Source: CAD feature listing. Evaluate the final solid. Frame: model axes, mm. A direction names the side the tool comes from. Round coordinates to 2 decimals unless told otherwise and drop trailing zeros. Write each loop counter-clockwise with the first axis right and the second up, starting at its lowest first coordinate (ties: lowest second). Pieces come first, ordered by that corner, then holes. Notation, with made-up numbers: M 7,-5.75 L 60,-5.75 A24 cw 60,24.25 Z; hole C 60.25,-7.5 d2. An arc over 180 degrees is marked long. Answer in a Markdown table with one row per item. Add a question column.
Item 1: Cut plane A-A on y = 2.25. Return loops of the section in (x, z), and give its area (3 significant figures).
Item 2: Cut plane B-B on z = -49. Return loops of the section in (x, y).
Item 3: Set-up query: faces 5 (the face through (-0.8, 15.1, -82.4)), 6 (the face through (-41.15, 14.93, -32.74)). Return all of +Z, -Z, +X, -X, +Y, -Y with unobstructed straight access to the full face (end or side cutting, diameter ignored); none if empty.
Item 4: Contact query for flat-ended pins moving along their axis: pin 1 (5 mm diameter, centred on y = 16, z = 35, fed in from -X); pin 2 (9.5 mm diameter, centred on x = 37.5, z = -37.5, fed in from +Y); pin 3 (11 mm diameter, centred on x = -37.5, z = -37.5, fed in from +Y). Output: stop coordinate, or through.
Item 5: Mould query, pull axis Z, two halves, no side actions, for faces 1 (the face through (-62.236, 5.07, -68.494)), 2 (the face through (36.87, 7.02, 36.67)), 3 (the face through (78.945, 5.07, -78.479)), 4 (the face through (-82.4, 15.1, 0.8)). Classes: released by +Z, released by -Z, zero draft, split by the parting line, or undercut.
Item 6: Material intervals for probe 1 along X at (y, z) = (15.75, -37.5); probe 2 along Z at (x, y) = (62.5, 8.25), sorted ascending.
from build123d import *

# Parameters (mm, degrees)
BASE_PLATE_SKETCH_175X175_W = 175
BASE_PLATE_SKETCH_175X175_H = 175
BASE_PLATE_DEPTH            = 20
CORNER_FILLETS_R30_R        = 30
EDGE_CHAMFER_10X45_SIZE     = 10
DOWEL_HOLES_12_INNER_D      = 12
DOWEL_HOLES_12_INNER_DEPTH  = 10
DOWEL_HOLES_12_INNER_TIP    = 3.605163714
DOWEL_HOLES_12_OUTER_D      = 12
DOWEL_HOLES_12_OUTER_DEPTH  = 10
DOWEL_HOLES_12_OUTER_TIP    = 3.605163714


with BuildPart() as part:
    # Base Plate Sketch 175x175 → Base Plate (new body)
    with BuildSketch(Plane(origin=(0, 0, 0), x_dir=(1, 0, 0), z_dir=(0, 1, 0))):
        Rectangle(BASE_PLATE_SKETCH_175X175_W, BASE_PLATE_SKETCH_175X175_H)
    extrude(amount=BASE_PLATE_DEPTH)

    # Corner Fillets R30
    corner_fillets_r30_edges = [part.edges().sort_by_distance(p)[0] for p in [
        (87.5, 10, 87.5),
        (-87.5, 10, 87.5),
        (-87.5, 10, -87.5),
        (87.5, 10, -87.5),
    ]]
    fillet(corner_fillets_r30_edges, radius=CORNER_FILLETS_R30_R)

    # Edge Chamfer 10x45
    edge_chamfer_10x45_edges = [part.edges().sort_by_distance(p)[0] for p in [
        (-87.5, 20, 0),
        (0, 20, -87.5),
        (87.5, 20, 0),
        (0, 20, 87.5),
        (-78.713203436, 20, 78.713203436),
        (78.713203436, 20, 78.713203436),
        (78.713203436, 20, -78.713203436),
        (-78.713203436, 20, -78.713203436),
    ]]
    chamfer(edge_chamfer_10x45_edges, length=EDGE_CHAMFER_10X45_SIZE)

    # Dowel Holes Ø12 Inner
    with Locations(Plane(origin=(-37.5, 20, -37.5), x_dir=(0, 0, 1), z_dir=(0, 1, 0))):
        with Locations((0, 0), (0, 75), (75, 75), (75, 0)):
            Hole(DOWEL_HOLES_12_INNER_D / 2, depth=DOWEL_HOLES_12_INNER_DEPTH)
            with Locations((0, 0, -(DOWEL_HOLES_12_INNER_DEPTH + DOWEL_HOLES_12_INNER_TIP / 2))):  # 118° drill point
                Cone(0, DOWEL_HOLES_12_INNER_D / 2, DOWEL_HOLES_12_INNER_TIP, mode=Mode.SUBTRACT)

    # Dowel Holes Ø12 Outer
    with Locations(Plane(origin=(-62.5, 0, 62.5), x_dir=(0, 0, -1), z_dir=(0, -1, 0))):
        with Locations((0, 0), (0, 125), (125, 125), (125, 0)):
            Hole(DOWEL_HOLES_12_OUTER_D / 2, depth=DOWEL_HOLES_12_OUTER_DEPTH)
            with Locations((0, 0, -(DOWEL_HOLES_12_OUTER_DEPTH + DOWEL_HOLES_12_OUTER_TIP / 2))):  # 118° drill point
                Cone(0, DOWEL_HOLES_12_OUTER_D / 2, DOWEL_HOLES_12_OUTER_TIP, mode=Mode.SUBTRACT)


solid = part.part
Results below:
| question | item | result |
|---|---|---|
| 1 | outline | M -87.5,-57.5 A30 ccw -57.5,-87.5 L 57.5,-87.5 A30 ccw 87.5,-57.5 L 87.5,57.5 A30 ccw 57.5,87.5 L -57.5,87.5 A30 ccw -87.5,57.5 Z; hole C -62.5,-62.5 d12; hole C -62.5,62.5 d12; hole C 62.5,-62.5 d12; hole C 62.5,62.5 d12 |
| 1 | area | 29,400 mm2 |
| 2 | outline | M -87.5,0 L 87.5,0 L 87.5,10 L 77.5,20 L -77.5,20 L -87.5,10 Z |
| 3 | face 5 | -Z, +X, -X, +Y |
| 3 | face 6 | +Y |
| 4 | pin 1 | x = -84 |
| 4 | pin 2 | y = 9.25 |
| 4 | pin 3 | y = 9.7 |
| 5 | face 1 | undercut |
| 5 | face 2 | undercut |
| 5 | face 3 | released by -Z |
| 5 | face 4 | zero draft |
| 6 | probe 1 | -81.75 to -43.5, -31.5 to 31.5, 43.5 to 81.75 |
| 6 | probe 2 | -87.08 to -68.5, -56.5 to 56.5, 68.5 to 87.08 |
